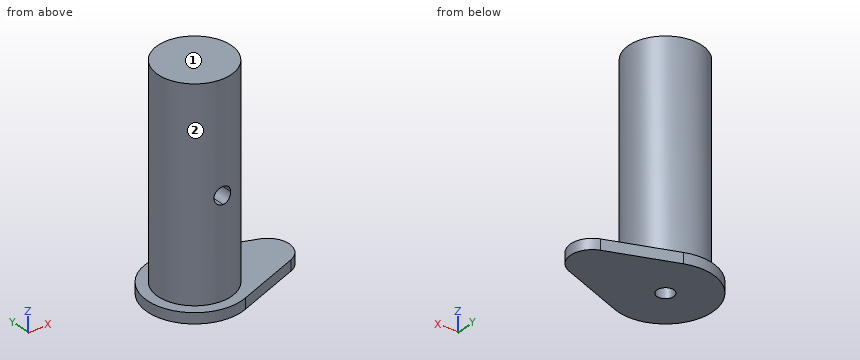
```python
from build123d import *

# Parameters (mm, degrees)
SKETCH_1_R          = 17.5
EXTRUDE_1_DEPTH     = 103
SKETCH_2_R          = 17.5
EXTRUDE_3_DEPTH     = 5
SKETCH_3_R          = 4
CUT_EXTRUDE_1_DEPTH = 70
CUT_EXTRUDE_2_DEPTH = 70


with BuildPart() as part:
    # Sketch 1 → Extrude 1 (new body)
    with BuildSketch(Plane.XY):
        Circle(SKETCH_1_R)
    extrude(amount=EXTRUDE_1_DEPTH)

    # Sketch 2 → Extrude 3 (add)
    with BuildSketch(Plane(origin=(0, 0, 0), x_dir=(-1, 0, 0), z_dir=(0, 0, -1))):
        with BuildLine():
            Line((-7.842143419, 21.089115358), (-38.590345949, 9.655168982))
            ThreePointArc((-38.590345949, 9.655168982), (-45.301110237, 0), (-38.590345949, -9.655168982))
            Line((-38.590345949, -9.655168982), (-7.842143419, -21.089115358))
            ThreePointArc((-7.842143419, -21.089115358), (22.5, 0), (-7.842143419, 21.089115358))
        make_face()
        Circle(SKETCH_2_R, mode=Mode.SUBTRACT)
    extrude(amount=-EXTRUDE_3_DEPTH)

    # Sketch 3 → Cut-Extrude 1 (cut)
    with BuildSketch(Plane(origin=(0, 0, 0), x_dir=(-1, 0, 0), z_dir=(0, 0, -1))):
        Circle(SKETCH_3_R)
    extrude(amount=-CUT_EXTRUDE_1_DEPTH, mode=Mode.SUBTRACT)

    # Sketch 4 → Cut-Extrude 2 (cut)
    with BuildSketch(Plane(origin=(0, 0, 0), x_dir=(1, 0, 0), z_dir=(0, 1, 0))):
        with BuildLine():
            Line((0, -51.5), (0, -55.5))
            ThreePointArc((0, -55.5), (2.828427125, -54.328427125), (4, -51.5))
            Line((4, -51.5), (0, -51.5))
        make_face()
        with BuildLine():
            Line((0, -47.5), (0, -51.5))
            Line((0, -51.5), (4, -51.5))
            ThreePointArc((4, -51.5), (2.828427125, -48.671572875), (0, -47.5))
        make_face()
        with BuildLine():
            ThreePointArc((0, -47.5), (-4, -51.5), (0, -55.5))
            Line((0, -55.5), (0, -51.5))
            Line((0, -51.5), (0, -47.5))
        make_face()
    extrude(amount=-CUT_EXTRUDE_2_DEPTH, mode=Mode.SUBTRACT)


solid = part.part
```
Geometry: final body of the model. Coordinates: model frame, mm. Face numbers are marked on the shaded views. A direction names the side the tool comes from. Coordinates: 2 decimals unless noted, no trailing zeros. Order: outer loops, then holes, each group sorted by start corner. A loop starts at its lowest first (then second) coordinate and runs counter-clockwise, first axis right, second up. Notation, with made-up numbers: (-31.5, 72.25) - (-26.5, 72.25) arc R20 cw to (-26.5, 91.25) - close; hole circle Ø9 at (45, -20). An arc over 180 degrees is marked (long way). Return JSON: item names as keys, results as strings. Group by question number.
1. Material intervals for line 1 along Z through (x, y) = (0, -11.5); line 2 along X through (y, z) = (0, 23), sorted ascending. Write a range as [from, to].
2. Cut plane C-C (y = 15.5). Output: boundary loops of the cut face in (x, z).
3. Set-up query: the marked faces 1 and 2. Return all of +Z, -Z, +X, -X, +Y, -Y with unobstructed straight access to the full face (end or side cutting, diameter ignored); none if empty.
4. Cut plane A-A (x = -14.5). Output: boundary loops of the cut face in (y, z).
5. Cut plane B-B (y = -11.5). Output: boundary loops of the cut face in (x, z).
6. Pin query (flat end, axial travel): pin 1 (6 mm diameter, centred on y = 7.5, z = 52, fed in from +X); pin 2 (6 mm diameter, centred on x = 0.5, z = 58, fed in from +Y); pin 3 (3 mm diameter, centred on y = 11, z = 89.5, fed in from +X). Return the tip coordinate at first contact, or that it passes through.
7. Cut plane D-D (x = 32). Output: boundary loops of the cut face in (y, z), plus the area to 3 significant figures.
Resolved:
{
 "1": {"line 1": "z = [0, 47.5], [55.5, 103]", "line 2": "x = [-17.5, -4], [4, 17.5]"},
 "2": {"outline": "(-16.31, 0) - (22.87, 0) - (22.87, 5) - (8.12, 5) - (8.12, 103) - (-8.12, 103) - (-8.12, 5) - (-16.31, 5) - close"},
 "3": {"face 1": "+Z, +X, -X, +Y, -Y", "face 2": "+Z"},
 "4": {"outline": "(-17.2, 0) - (17.2, 0) - (17.2, 5) - (9.8, 5) - (9.8, 103) - (-9.8, 103) - (-9.8, 5) - (-17.2, 5) - close"},
 "5": {"outline": "(-19.34, 0) - (33.63, 0) - (33.63, 5) - (13.19, 5) - (13.19, 103) - (-13.19, 103) - (-13.19, 5) - (-19.34, 5) - close; hole circle Ø8 at (0, 51.5)"},
 "6": {"pin 1": "stops at x = 16.91", "pin 2": "stops at y = 17.5", "pin 3": "stops at x = 14.7"},
 "7": {"outline": "(-12.11, 0) - (12.11, 0) - (12.11, 5) - (-12.11, 5) - close", "area": "121 mm²"}
}
